The figure shows three views and two pictorial views of one solid part (mm, origin at its lowest corner). Answer the questions. Coordinates: 2 decimals unless noted, no trailing zeros. Loops run counter-clockwise (first coordinate to the right, second up) from the corner with the lowest first, then second, coordinate; pieces in that order, holes last. Notation, with made-up numbers: (54, 37) - (105, 37) arc R19 cw to (105, 70) - close; hole circle Ø2 at (4, 39). An arc over 180 degrees is marked (long way). Return JSON: item names as keys, results as strings. Group by question number.
1. Section A-A (x = 27.75) is taken. Write down the section's boundary in (y, z), and give its area (3 significant figures).
2. The mould has two halves that part along X. Classify the marked faces 1, 2 and 3: pulls with the +X half, pulls with the -X half, needs draft (parallel to the pull), parting line crosses it, or undercut.
3. Each of these flat-tipped pins is pushed along its axis until it touches: P1, Ø2, axis at x = 33, y = 22, coming from the +Z side; P2, Ø2, axis at x = 26.5, z = 22, coming from the +Y side; P3, Ø10, axis at x = 41, y = 6.5, coming from the -Z side; P4, Ø6, axis at y = 5, z = 6, coming from the +X side. Where does it stop, or does it pass through?
4. Section B-B (z = 27.75) is taken. Write down the section's boundary in (x, y).
5. Find the intervals of material crossed by line 1 along Z through (x, y) = (28, 34.5); line 2 along Y through (x, z) = (32, 36.5), in increasing order.
6. Section C-C (y = 33) is taken. Write down the section's boundary in (x, z).
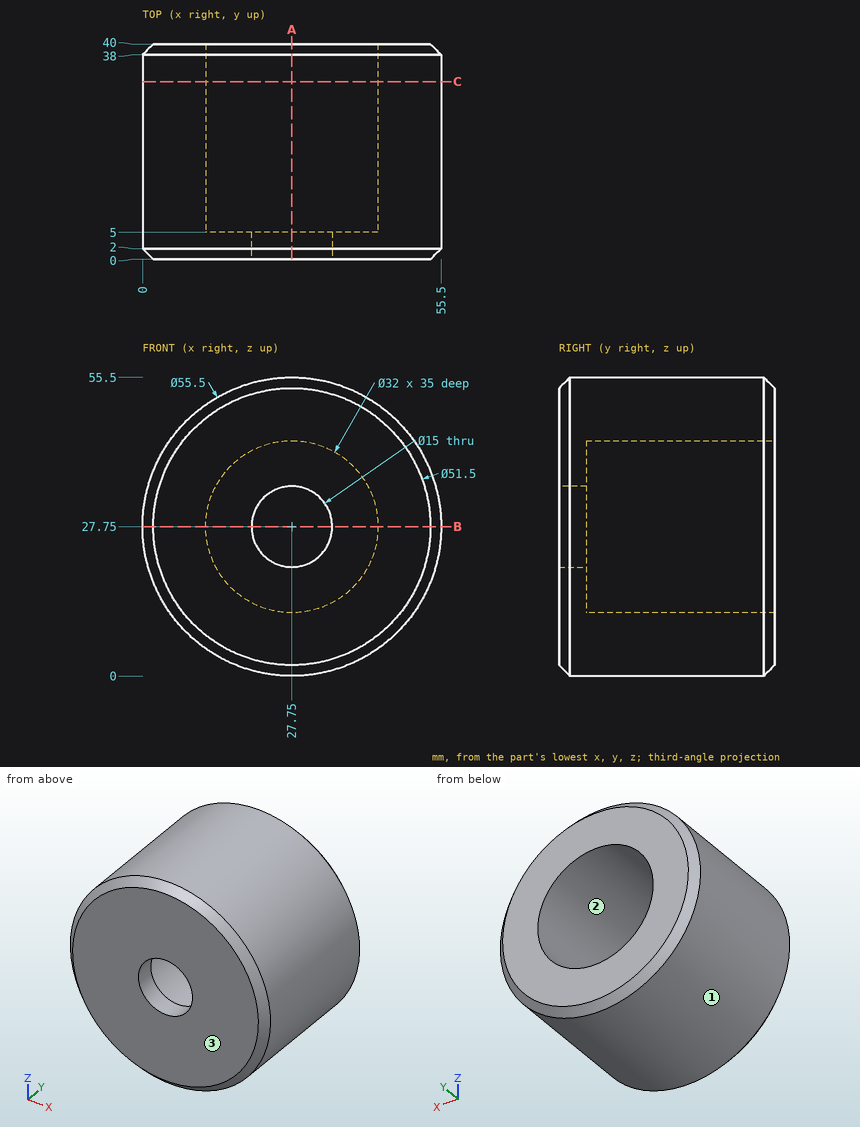
The answers:
{
 "1": {"outline": "(0, 2) - (2, 0) - (38, 0) - (40, 2) - (40, 11.75) - (5, 11.75) - (5, 20.25) - (0, 20.25) - close; (0, 35.25) - (5, 35.25) - (5, 43.75) - (40, 43.75) - (40, 53.5) - (38, 55.5) - (2, 55.5) - (0, 53.5) - close", "area": "1,020 mm2"},
 "2": {"face 1": "parting line crosses it", "face 2": "undercut", "face 3": "needs draft"},
 "3": {"P1": "stops at z = 55.17", "P2": "passes through", "P3": "stops at z = 1.25", "P4": "stops at x = 48.21"},
 "4": {"outline": "(0, 2) - (2, 0) - (20.25, 0) - (20.25, 5) - (11.75, 5) - (11.75, 40) - (2, 40) - (0, 38) - close; (35.25, 0) - (53.5, 0) - (55.5, 2) - (55.5, 38) - (53.5, 40) - (43.75, 40) - (43.75, 5) - (35.25, 5) - close"},
 "5": {"line 1": "z = 0 to 11.75, 43.75 to 55.5", "line 2": "y = 0 to 5"},
 "6": {"outline": "circle Ø55.5 at (27.75, 27.75); hole circle Ø32 at (27.75, 27.75)"}
}
